```python
from build123d import *

# Parameters (mm, degrees)
SKETCH_1_W             = 75
SKETCH_1_H             = 39.5
EXTRUDE_1_DEPTH        = 34
SKETCH_2_R             = 16.5
CUT_EXTRUDE_1_DEPTH    = 55.335186574
SKETCH_3_W             = 20
SKETCH_3_H             = 4.375595252
CUT_EXTRUDE_2_DEPTH    = 55.335186574
HOLE_WIZARD_M8_1_D     = 6.8
HOLE_WIZARD_M8_1_DEPTH = 19.75
HOLE_WIZARD_M8_1_TIP   = 2.042926105
CHAMFER_1_SIZE         = 5
CHAMFER_2_SIZE         = 1
HOLE_WIZARD_M6_1_D     = 5
HOLE_WIZARD_M6_1_DEPTH = 15
HOLE_WIZARD_M6_1_TIP   = 1.502151548


with BuildPart() as part:
    # 草图1 → 凸台-拉伸1 (new body)
    with BuildSketch(Plane.XY):
        Rectangle(SKETCH_1_W, SKETCH_1_H)
    extrude(amount=EXTRUDE_1_DEPTH)

    # 草图2 → 切除-拉伸1 (cut, through all)
    with BuildSketch(Plane.XY.offset(34)):
        with Locations((0, -2.25)):
            Circle(SKETCH_2_R)
    extrude(amount=-CUT_EXTRUDE_1_DEPTH, mode=Mode.SUBTRACT)

    # 草图3 → 切除-拉伸2 (cut, through all)
    with BuildSketch(Plane.XY.offset(34)):
        with Locations((0, -17.562202374)):
            Rectangle(SKETCH_3_W, SKETCH_3_H)
    extrude(amount=-CUT_EXTRUDE_2_DEPTH, mode=Mode.SUBTRACT)

    # M8 螺纹孔1
    with Locations(Plane(origin=(0, 19.75, 0), x_dir=(1, 0, 0), z_dir=(0, 1, 0))):
        with Locations((-27.5, -7), (-27.5, -27), (27.5, -27), (27.5, -7)):
            Hole(HOLE_WIZARD_M8_1_D / 2, depth=HOLE_WIZARD_M8_1_DEPTH)
            with Locations((0, 0, -(HOLE_WIZARD_M8_1_DEPTH + HOLE_WIZARD_M8_1_TIP / 2))):  # 118° drill point
                Cone(0, HOLE_WIZARD_M8_1_D / 2, HOLE_WIZARD_M8_1_TIP, mode=Mode.SUBTRACT)

    # 倒角1
    chamfer_1_edges = [part.edges().sort_by_distance(p)[0] for p in [
        (37.5, -19.75, 17),
        (-37.5, -19.75, 17),
    ]]
    chamfer(chamfer_1_edges, length=CHAMFER_1_SIZE)

    # 倒角2
    chamfer_2_edges = [part.edges().sort_by_distance(p)[0] for p in [
        (-37.5, 2.5, 34),
        (0, 14.25, 0),
        (0, 14.25, 34),
        (-37.5, 2.5, 0),
        (37.5, 2.5, 0),
        (37.5, 2.5, 34),
    ]]
    chamfer(chamfer_2_edges, length=CHAMFER_2_SIZE)

    # M6 螺纹孔1
    with Locations(Plane.XY.offset(34)):
        with Locations((-18.186533479, 8.25), (-18.186533479, -12.75), (18.186533479, 8.25), (18.186533479, -12.75)):
            Hole(HOLE_WIZARD_M6_1_D / 2, depth=HOLE_WIZARD_M6_1_DEPTH)
            with Locations((0, 0, -(HOLE_WIZARD_M6_1_DEPTH + HOLE_WIZARD_M6_1_TIP / 2))):  # 118° drill point
                Cone(0, HOLE_WIZARD_M6_1_D / 2, HOLE_WIZARD_M6_1_TIP, mode=Mode.SUBTRACT)


solid = part.part
```
For this review, take the finished solid that the model builds, in its own axes (mm). A direction names the side the tool comes from. Coordinates: 2 decimals unless noted, no trailing zeros. Loops run counter-clockwise (first coordinate to the right, second up) from the corner with the lowest first, then second, coordinate; pieces in that order, holes last.
1. Add section C-C, the plane z = 11.5. Give the boundary of the cut face in (x, y).
2. For faces 1 (the flat face through (34.97, -17.28, 16.76)), 2 (the cylindrical face through (-17.64, 5.81, 26.4)), 3 (the flat face through (-10, -18, 17)), list the 3-axis set-ups (+Z, -Z, +X, -X, +Y, -Y) from which the entire face can be reached by the end or side of a thin tool; tool diameter is ignored.
3. Add section D-D, the plane x = 0. Give the boundary of the cut face in (y, z).
4. Mouldability with a two-part tool opening along Z and no side actions: class faces 4 (the conical face through (0.59, 14.4, 0.84)), 5 (the cylindrical face through (20.17, -14.27, 26.4)), 6 (the cylindrical face through (24.257, 9.737, 25.979)) as +Z half, -Z half, draft (parallel to the pull), parting line (faces both ways), or undercut.
5. Insertion check: P1, Ø6, axis at x = -27.5, z = 7, coming from the +Y side; P2, Ø5, axis at y = -18.5, z = 19.5, coming from the +X side; P3, Ø3.5, axis at y = -18, z = 11, coming from the -X side. Each pin has a flat end and moves straight along its axis. Give the tip position at first contact, or say it passes through.
6. Add section A-A, the plane z = 21.5. Give the boundary of the cut face in (x, y).
7. Add section B-B, the plane y = 17.5. Give the boundary of the cut face in (x, z).
8. For line 1 (Z direction, x = 27.5, y = 9.5); line 2 (X direction, y = 10.5, z = 4); line 3 (X direction, y = 10.5, z = 27), list the stretches that pass through material, from the lowest coordinate up.
Result:
1. outline: (-37.5, -14.75) - (-32.5, -19.75) - (-10, -19.75) - (-10, -15.37) arc R16.5 cw (long way) to (10, -15.37) - (10, -19.75) - (32.5, -19.75) - (37.5, -14.75) - (37.5, 19.75) - (-37.5, 19.75) - close
2. face 1: +Z, -Z, +X, -Y
2. face 2: +Z
2. face 3: +Z, -Z, -Y
3. outline: (14.25, 1) - (15.25, 0) - (19.75, 0) - (19.75, 34) - (15.25, 34) - (14.25, 33) - close
4. face 4: -Z half
4. face 5: draft
4. face 6: undercut
5. P1: stops at y = -0.24
5. P2: stops at x = 36.25
5. P3: stops at x = -36
6. outline: (-37.5, -14.75) - (-32.5, -19.75) - (-10, -19.75) - (-10, -15.37) arc R16.5 cw (long way) to (10, -15.37) - (10, -19.75) - (32.5, -19.75) - (37.5, -14.75) - (37.5, 19.75) - (-37.5, 19.75) - close; hole circle Ø5 at (-18.19, -12.75); hole circle Ø5 at (-18.19, 8.25); hole circle Ø5 at (18.19, -12.75); hole circle Ø5 at (18.19, 8.25)
7. outline: (-37.5, 1) - (-36.5, 0) - (36.5, 0) - (37.5, 1) - (37.5, 33) - (36.5, 34) - (-36.5, 34) - (-37.5, 33) - close; hole circle Ø6.8 at (-27.5, 7); hole circle Ø6.8 at (-27.5, 27); hole circle Ø6.8 at (27.5, 7); hole circle Ø6.8 at (27.5, 27)
8. line 1: z = 0 to 3.6, 10.4 to 23.6, 30.4 to 34
8. line 2: x = -37.5 to -29.1, -25.9 to -10.47, 10.47 to 25.9, 29.1 to 37.5
8. line 3: x = -37.5 to -30.9, -24.1 to -19.28, -17.1 to -10.47, 10.47 to 17.1, 19.28 to 24.1, 30.9 to 37.5
